Verification items for the finished model (mm, model axes). Face numbers are marked on the shaded views. A direction names the side the tool comes from. Give positions to 0.01 mm unless a question says otherwise; leave off trailing zeros. Order: outer loops, then holes, each group sorted by start corner. A loop starts at its lowest first (then second) coordinate and runs counter-clockwise, first axis right, second up. Notation, with made-up numbers: M 34,50 L 43,50 A29 ccw 43,71 Z; hole C 36,67.5 d6. An arc over 180 degrees is marked long. Answer as a JSON object with one key per item and string values.
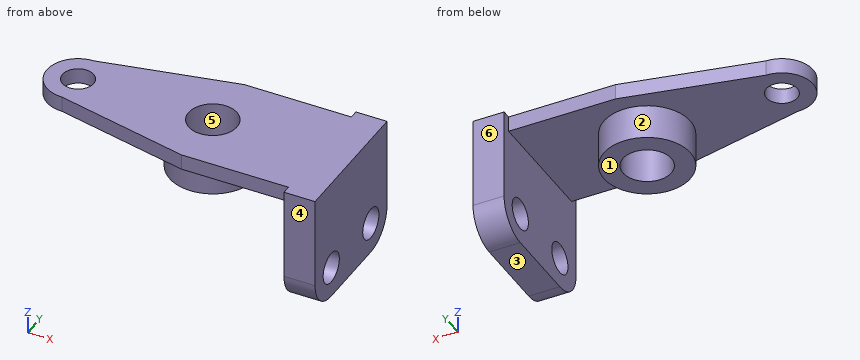
```python
from build123d import *

# Parameters (mm, degrees)
BASE_PLATE_DEPTH              = 9
END_HOLE_18_SKETCH_R          = 9
END_HOLE_18_DEPTH             = 9
PIVOT_BOSS_50_SKETCH_R        = 25
PIVOT_BOSS_50_DEPTH           = 20
PIVOT_BORE_28_SKETCH_R        = 14
PIVOT_BORE_28_DEPTH           = 126.227792442
MOUNTING_BLOCK_DEPTH          = 18
MOUNTING_HOLES_2X_18_SKETCH_R = 9
MOUNTING_HOLES_2X_18_DEPTH    = 18


with BuildPart() as part:
    # Base Plate Profile Sketch → Base Plate (new body)
    with BuildSketch(Plane.XY):
        with BuildLine():
            Line((-78, 53), (0, 70))
            Line((0, 70), (69.753049234, 70))
            ThreePointArc((69.753049234, 70), (75.45392636, 71.316678554), (80, 75))
            Line((80, 75), (80, -5))
            ThreePointArc((80, -5), (75.45392636, -1.316678554), (69.753049234, 0))
            Line((69.753049234, 0), (0, 0))
            Line((0, 0), (-78, 17))
            ThreePointArc((-78, 17), (-96, 35), (-78, 53))
        make_face()
    extrude(amount=BASE_PLATE_DEPTH)

    # End Hole Ø18 Sketch → End Hole Ø18 (cut)
    with BuildSketch(Plane(origin=(0, 0, 0), x_dir=(-1, 0, 0), z_dir=(0, 0, -1))):
        with Locations((78, 35)):
            Circle(END_HOLE_18_SKETCH_R)
    extrude(amount=-END_HOLE_18_DEPTH, mode=Mode.SUBTRACT)

    # Pivot Boss Ø50 Sketch → Pivot Boss Ø50 (add)
    with BuildSketch(Plane(origin=(0, 0, 0), x_dir=(-1, 0, 0), z_dir=(0, 0, -1))):
        with Locations(Location((0, 35, 0), (0, 0, 180))):
            Circle(PIVOT_BOSS_50_SKETCH_R)
    extrude(amount=PIVOT_BOSS_50_DEPTH)

    # Pivot Bore Ø28 Sketch → Pivot Bore Ø28 (cut, through all)
    with BuildSketch(Plane(origin=(0, 0, -20), x_dir=(-1, 0, 0), z_dir=(0, 0, -1))):
        with Locations((0, 35)):
            Circle(PIVOT_BORE_28_SKETCH_R)
    extrude(amount=-PIVOT_BORE_28_DEPTH, mode=Mode.SUBTRACT)

    # Mounting Block Sketch → Mounting Block (add)
    with BuildSketch(Plane(origin=(80, 0, 0), x_dir=(0, 0, -1), z_dir=(1, 0, 0))):
        with BuildLine():
            Line((-9, 75), (44, 75))
            ThreePointArc((44, 75), (56.727922061, 69.727922061), (62, 57))
            Line((62, 57), (62, 13))
            ThreePointArc((62, 13), (56.727922061, 0.272077939), (44, -5))
            Line((44, -5), (-9, -5))
            Line((-9, -5), (-9, 75))
        make_face()
    extrude(amount=-MOUNTING_BLOCK_DEPTH)

    # Mounting Holes 2xØ18 Sketch → Mounting Holes 2xØ18 (cut)
    with BuildSketch(Plane(origin=(80, 0, 0), x_dir=(0, 0, -1), z_dir=(1, 0, 0))):
        with Locations((44, 57)):
            Circle(MOUNTING_HOLES_2X_18_SKETCH_R)
        with Locations((44, 13)):
            Circle(MOUNTING_HOLES_2X_18_SKETCH_R)
    extrude(amount=-MOUNTING_HOLES_2X_18_DEPTH, mode=Mode.SUBTRACT)


solid = part.part
```
Q1. Section check C-C on x = 35.5. Record the cut outline in (y, z).
Resolved:
{"outline": "M 0,0 L 70,0 L 70,9 L 0,9 Z"}
Q2. Release check for a two-part mould opening along Y. For the marked faces 4, 5 and 6 record: +Y half, -Y half, draft (parallel to the pull), parting line (faces both ways), or undercut.
Resolved:
{"face 4": "-Y half", "face 5": "undercut", "face 6": "+Y half"}
Q3. Section check B-B on y = 19. Record the cut outline in (x, z), then the cut area to 3 significant figures.
Resolved:
{"outline": "M -86.25,0 L -19.21,0 L -19.21,-20 L 19.21,-20 L 19.21,0 L 62,0 L 62,-37.29 L 80,-37.29 L 80,9 L -86.25,9 Z; M 62,-62 L 80,-62 L 80,-50.71 L 62,-50.71 Z", "area": "3,140 mm²"}
Q4. Tool access check on the marked faces 1, 2 and 3. Record the directions out of +Z, -Z, +X, -X, +Y, -Y that give a thin tool (end or side, any length) a straight path to the whole face; none if there is none.
Resolved:
{"face 1": "-Z, -X, +Y, -Y", "face 2": "-Z", "face 3": "-Z, +X, -X, +Y, -Y"}
Q5. Section check D-D on z = -56.5. Record the cut outline in (x, y), then the cut area to 3 significant figures.
Resolved:
{"outline": "M 62,0.05 L 80,0.05 L 80,69.95 L 62,69.95 Z", "area": "1,260 mm²"}
Q6. Section check A-A on y = 35. Record the cut outline in (x, z), then the cut area to 3 significant figures.
Resolved:
{"outline": "M -96,0 L -87,0 L -87,9 L -96,9 Z; M -69,0 L -25,0 L -25,-20 L -14,-20 L -14,9 L -69,9 Z; M 14,-20 L 25,-20 L 25,0 L 62,0 L 62,-62 L 80,-62 L 80,9 L 14,9 Z", "area": "2,730 mm²"}
Q7. Gauge pin test, flat ends, axial feed: pin 1 Ø8 at (x, y) = (-52.5, 24.5) entering from -Z; pin 2 Ø4.5 at (x, z) = (27, 3.5) entering from +Y; pin 3 Ø2 at (y, z) = (30.5, -35.5) entering from -X; pin 4 Ø3 at (y, z) = (51, -48) entering from -X. Record the tip position at first contact, or that the pin passes through.
Resolved:
{"pin 1": "stops at z = 0", "pin 2": "stops at y = 70", "pin 3": "stops at x = 62", "pin 4": "passes through"}
Q8. Material ranges on L1, parallel to Y at x = 68.5, z = -44; L2, parallel to Y at x = 70, z = -36.5; L3, parallel to X at y = 30.5, z = -31, recorded low to high.
Resolved:
{"L1": "y = -5 to 4, 22 to 48, 66 to 75", "L2": "y = -5 to 8.03, 17.97 to 52.03, 61.97 to 75", "L3": "x = 62 to 80"}
